```python
from build123d import *

# Parameters (mm, degrees)
SKETCH1_R           = 10
BOSS_EXTRUDE1_DEPTH = 5
SKETCH2_R           = 11.5
BOSS_EXTRUDE2_DEPTH = 3
SKETCH3_R           = 10
BOSS_EXTRUDE3_DEPTH = 20
SKETCH4_R           = 5
BOSS_EXTRUDE4_DEPTH = 30
SKETCH5_R           = 2.5
BOSS_EXTRUDE5_DEPTH = 10


with BuildPart() as part:
    # Sketch1 → Boss-Extrude1 (new body)
    with BuildSketch(Plane.XY):
        Circle(SKETCH1_R)
    extrude(amount=BOSS_EXTRUDE1_DEPTH)

    # Sketch2 → Boss-Extrude2 (add)
    with BuildSketch(Plane.XY.offset(5)):
        Circle(SKETCH2_R)
    extrude(amount=BOSS_EXTRUDE2_DEPTH)

    # Sketch3 → Boss-Extrude3 (add)
    with BuildSketch(Plane.XY.offset(8)):
        Circle(SKETCH3_R)
    extrude(amount=BOSS_EXTRUDE3_DEPTH)

    # Sketch4 → Boss-Extrude4 (add)
    with BuildSketch(Plane.XY.offset(28)):
        Circle(SKETCH4_R)
    extrude(amount=BOSS_EXTRUDE4_DEPTH)

    # Sketch5 → Boss-Extrude5 (add)
    with BuildSketch(Plane.XY.offset(58)):
        Circle(SKETCH5_R)
    extrude(amount=BOSS_EXTRUDE5_DEPTH)


solid = part.part
```
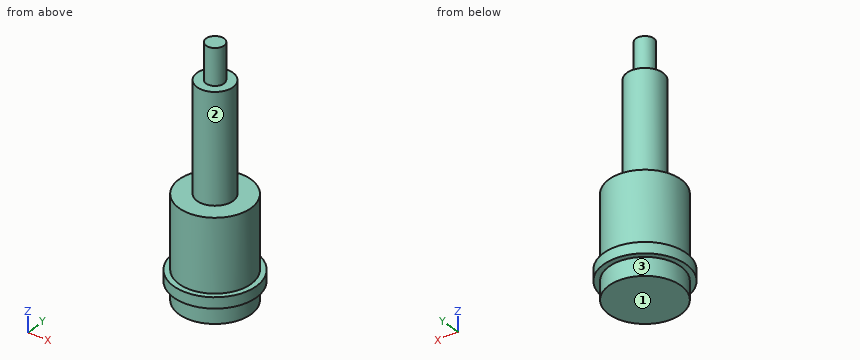
The listing builds one solid part. Answer for the finished solid, in the listing's coordinates (mm). Face numbers are marked on the shaded views. A direction names the side the tool comes from. Round coordinates to 2 decimals unless told otherwise and drop trailing zeros. Loops run counter-clockwise (first coordinate to the right, second up) from the corner with the lowest first, then second, coordinate; pieces in that order, holes last.
Q1. Section C-C, the plane z = 27 is taken. Determine the outline of the cut face in (x, y).
Q2. Which of the six approach directions +Z, -Z, +X, -X, +Y, -Y give full straight-line access (tool end or side, diameter ignored) to the marked faces 1, 2 and 3?
Q3. Section D-D, the plane y = -7 is taken. Determine the outline of the cut face in (x, z).
Q4. Section B-B, the plane x = 1.5 is taken. Determine the outline of the cut face in (y, z).
Q5. Given pin 1 Ø8 at (x, z) = (1.5, 37.5) entering from +Y; pin 2 Ø2 at (y, z) = (-2.5, 12.5) entering from -X; pin 3 Ø5 at (x, z) = (-2.5, 24.5) entering from -Y, each flat-ended and moving along its own axis, determine where each tip first touches the part or whether it passes through.
Q6. Find the intervals of material crossed by line 1 (X direction, y = -0.5, z = 23.5); line 2 (Z direction, x = -3.5, y = 9.5); line 3 (Z direction, x = -5.5, y = -8), in increasing order.
Q7. Section A-A, the plane y = 0 is taken. Determine the outline of the cut face in (x, z), then the cut area to 3 significant figures.
Completed:
1. outline: circle Ø20 at (0, 0)
2. face 1: -Z, +X, -X, +Y, -Y
2. face 2: +Z
2. face 3: -Z
3. outline: (-9.12, 5) - (-7.14, 5) - (-7.14, 0) - (7.14, 0) - (7.14, 5) - (9.12, 5) - (9.12, 8) - (7.14, 8) - (7.14, 28) - (-7.14, 28) - (-7.14, 8) - (-9.12, 8) - close
4. outline: (-11.4, 5) - (-9.89, 5) - (-9.89, 0) - (9.89, 0) - (9.89, 5) - (11.4, 5) - (11.4, 8) - (9.89, 8) - (9.89, 28) - (4.77, 28) - (4.77, 58) - (2, 58) - (2, 68) - (-2, 68) - (-2, 58) - (-4.77, 58) - (-4.77, 28) - (-9.89, 28) - (-9.89, 8) - (-11.4, 8) - close
5. pin 1: stops at y = 5
5. pin 2: stops at x = -9.89
5. pin 3: stops at y = -10
6. line 1: x = -9.99 to 9.99
6. line 2: z = 5 to 8
6. line 3: z = 0 to 28
7. outline: (-11.5, 5) - (-10, 5) - (-10, 0) - (10, 0) - (10, 5) - (11.5, 5) - (11.5, 8) - (10, 8) - (10, 28) - (5, 28) - (5, 58) - (2.5, 58) - (2.5, 68) - (-2.5, 68) - (-2.5, 58) - (-5, 58) - (-5, 28) - (-10, 28) - (-10, 8) - (-11.5, 8) - close
7. area: 919 mm2
